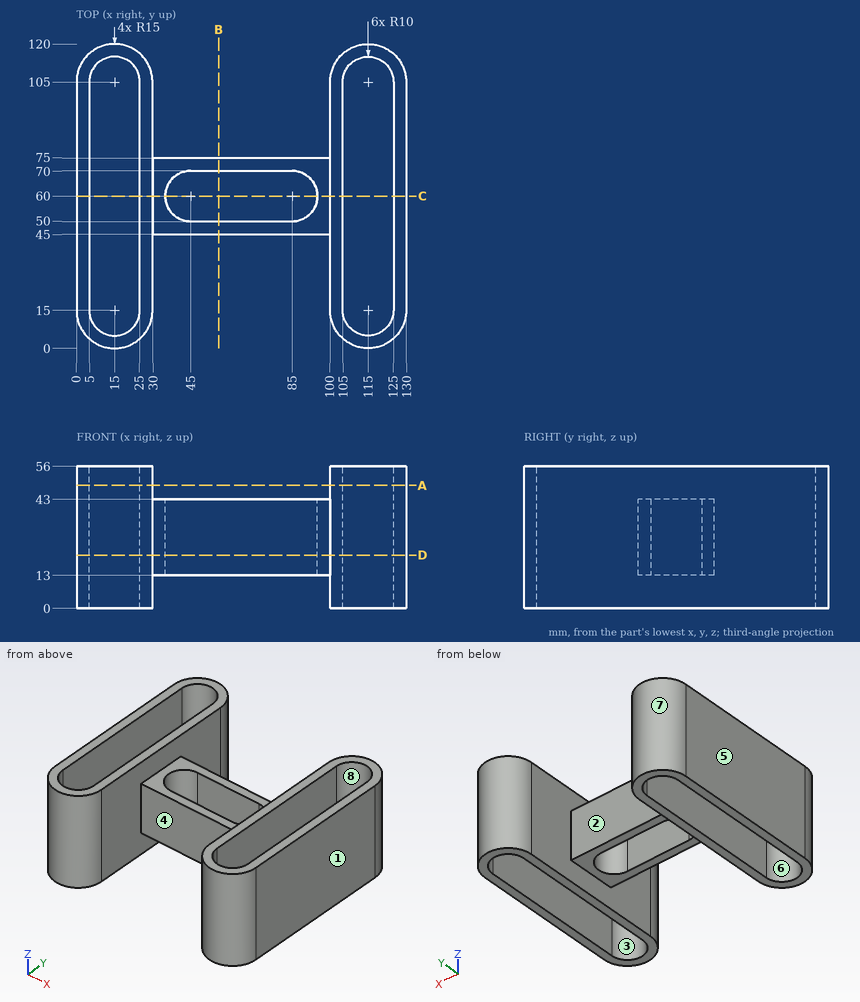
Here's the drawing with two shaded views (mm, measured from the low corner). I have some questions. A direction names the side the tool comes from. Give positions to 0.01 mm unless a question says otherwise; leave off trailing zeros. Loops run counter-clockwise (first coordinate to the right, second up) from the corner with the lowest first, then second, coordinate; pieces in that order, holes last. Notation, with made-up numbers: M 33,-6.5 L 49,-6.5 A32 cw 49,22.5 Z; hole C 66.25,56 d9. An arc over 180 degrees is marked long. Use one line per item in the form item = value. Start each with the question number.
(1) Please list where these lines run through material, in increasing order: line 1 (X direction, y = 100.5, z = 23.5); line 2 (X direction, y = 55, z = 17); line 3 (Y direction, x = 15.5, z = 3).
(2) I want a section at D-D, the plane z = 21. Write out the boundary of the cut face in (x, y), and give its area (3 significant figures).
(3) I want a section at A-A, the plane z = 48.5. Write out the boundary of the cut face in (x, y), and give its area (3 significant figures).
(4) On a 3-axis mill with a long thin cutter (end or side, diameter ignored), from which of +Z, -Z, +X, -X, +Y, -Y can I reach the whole of each face in a straight line? I mean the marked faces 1, 2, 3 and 4. Say none if no direction works.
(5) I'm going to push flat-ended pins straight in: P1, Ø9, axis at x = 69.5, z = 32, coming from the +Y side; P2, Ø8, axis at x = 78, y = 73.5, coming from the +Z side; P3, Ø9, axis at x = 49, y = 63.5, coming from the +Z side; P4, Ø15, axis at x = 57, z = 29.5, coming from the -Y side. Where does each tip first touch, or does it pass through?
(6) Thinking about a two-plate mould opening in Y: for the marked faces 5, 6, 7 and 8, which applies, released by +Y, released by -Y, zero draft, split by the parting line, or undercut?
(7) I want a section at B-B, the plane x = 56. Write out the boundary of the cut face in (y, z).
(8) I want a section at C-C, the plane y = 60. Write out the boundary of the cut face in (x, z).
Worked out:
q1.line_1 = 0 to 5, 25 to 30, 100 to 105, 125 to 130
q1.line_2 = 0 to 5, 25 to 36.34, 93.66 to 105, 125 to 130
q1.line_3 = 0.01 to 5.01, 114.99 to 119.99
q2.outline = M 0,15 A15 ccw 30,15 L 30,45 L 100,45 L 100,15 A15 ccw 130,15 L 130,105 A15 ccw 100,105 L 100,75 L 30,75 L 30,105 A15 ccw 0,105 Z; hole M 5,15 A10 ccw 25,15 L 25,105 A10 ccw 5,105 Z; hole M 45,50 L 85,50 A10 ccw 85,70 L 45,70 A10 ccw Z; hole M 105,15 A10 ccw 125,15 L 125,105 A10 ccw 105,105 Z
q2.area = 3,570 mm²
q3.outline = M 0,15 A15 ccw 30,15 L 30,105 A15 ccw 0,105 Z; M 100,15 A15 ccw 130,15 L 130,105 A15 ccw 100,105 Z; hole M 5,15 A10 ccw 25,15 L 25,105 A10 ccw 5,105 Z; hole M 105,15 A10 ccw 125,15 L 125,105 A10 ccw 105,105 Z
q3.area = 2,590 mm²
q4.face_1 = +Z, -Z, +X, +Y, -Y
q4.face_2 = +Z, -Z, +Y
q4.face_3 = +Z, -Z
q4.face_4 = +Z, -Z, -Y
q5.P1 = 75
q5.P2 = 43
q5.P3 = through
q5.P4 = 45
q6.face_5 = zero draft
q6.face_6 = undercut
q6.face_7 = released by +Y
q6.face_8 = undercut
q7.outline = M 45,13 L 50,13 L 50,43 L 45,43 Z; M 70,13 L 75,13 L 75,43 L 70,43 Z
q8.outline = M 0,0 L 5,0 L 5,56 L 0,56 Z; M 25,0 L 30,0 L 30,13 L 35,13 L 35,43 L 30,43 L 30,56 L 25,56 Z; M 95,13 L 100,13 L 100,0 L 105,0 L 105,56 L 100,56 L 100,43 L 95,43 Z; M 125,0 L 130,0 L 130,56 L 125,56 Z
